Geometry check sheet. Reference: the model listing, model coordinates, mm. Give positions to 0.01 mm unless a question says otherwise; leave off trailing zeros. Order: outer loops, then holes, each group sorted by start corner. A loop starts at its lowest first (then second) coordinate and runs counter-clockwise, first axis right, second up.
```python
from build123d import *

# Parameters (mm, degrees)
SKETCH1_W           = 28
SKETCH1_H           = 28
SKETCH1_R           = 5
BOSS_EXTRUDE1_DEPTH = 30
M12_TAPPED_HOLE1_D  = 10.2


with BuildPart() as part:
    # Sketch1 → Boss-Extrude1 (new body)
    with BuildSketch(Plane(origin=(0, 0, 0), x_dir=(1, 0, 0), z_dir=(0, 1, 0))):
        Rectangle(SKETCH1_W, SKETCH1_H)
        with Locations(Location((0, 0, 0), (0, 0, 270))):
            Circle(SKETCH1_R, mode=Mode.SUBTRACT)
    extrude(amount=BOSS_EXTRUDE1_DEPTH)

    # M12 Tapped Hole1 (through all)
    with Locations(Plane(origin=(0, 30, 0), x_dir=(1, 0, 0), z_dir=(0, 1, 0))):
        with Locations((0, 0)):
            Hole(M12_TAPPED_HOLE1_D / 2)


solid = part.part
```
Q1. Cross-section at A-A, the plane x = 0. Record the boundary of the cut face in (y, z).
Q2. Release check for a two-part mould opening along Z. For faces 1 (the face through (-6, 30, 0)), 2 (the face through (0, 15, -14)), 3 (the face through (-2.4, 14.8, 4.5)) record: pulls with the +Z half, pulls with the -Z half, needs draft (parallel to the pull), parting line crosses it, or undercut.
Q3. Thickness scan on L1, parallel to Z at x = 0, y = 21; L2, parallel to Z at x = -3, y = 18; L3, parallel to X at y = 6, z = -2. Record the ranges inside material, lowest first.
Q4. Cross-section at C-C, the plane z = 3.75. Record the boundary of the cut face in (x, y).
Q5. Cross-section at B-B, the plane y = 23.5. Record the boundary of the cut face in (x, z), and give its area (3 significant figures).
Q6. Gauge pin test, flat end, axial feed: P1, Ø13.5, axis at x = 0, z = 0, coming from the -Y side. Record the tip position at first contact, or that the pin passes through.
Answers follow:
1. outline: (0, -14) - (30, -14) - (30, -5.1) - (0, -5.1) - close; (0, 5.1) - (30, 5.1) - (30, 14) - (0, 14) - close
2. face 1: needs draft
2. face 2: pulls with the -Z half
2. face 3: undercut
3. L1: z = -14 to -5.1, 5.1 to 14
3. L2: z = -14 to -4.12, 4.12 to 14
3. L3: x = -14 to -4.69, 4.69 to 14
4. outline: (-14, 0) - (-3.46, 0) - (-3.46, 30) - (-14, 30) - close; (3.46, 0) - (14, 0) - (14, 30) - (3.46, 30) - close
5. outline: (-14, -14) - (14, -14) - (14, 14) - (-14, 14) - close; hole circle Ø10.2 at (0, 0)
5. area: 702 mm2
6. P1: stops at y = 0
